Check sheet for the modelled part. Datum: model origin and axes. Units: mm. Face numbers are marked on the shaded views. A direction names the side the tool comes from. Round coordinates to 2 decimals unless told otherwise and drop trailing zeros. Loops run counter-clockwise (first coordinate to the right, second up) from the corner with the lowest first, then second, coordinate; pieces in that order, holes last. Notation, with made-up numbers: M -6,42 L 17,42 A25 ccw 17,63 Z; hole C 49,9.5 d6. An arc over 180 degrees is marked long. One line per question, with ' | ' between items. Start each with the question number.
(1) Section check C-C (y = 16.5). Record the boundary of the cut face in (x, z), and give its area (3 significant figures).
(2) Go/stop test with flat-tipped pins: P1, Ø0.9, axis at y = 39, z = 4, coming from the -X side; P2, Ø4, axis at y = 20, z = 3, coming from the +X side; P3, Ø1.5, axis at y = 24.5, z = 6.5, coming from the +X side. Record where each tip stops, or that it passes through.
(3) Section check B-B (x = 0). Record the boundary of the cut face in (y, z).
(4) Section check A-A (z = 0). Record the boundary of the cut face in (x, y), and give its area (3 significant figures).
(5) Section check D-D (y = 33). Record the boundary of the cut face in (x, z).
(6) Tool access check on the marked faces 4 and 5. Record the directions out of +Z, -Z, +X, -X, +Y, -Y that give a thin tool (end or side, any length) a straight path to the whole face; none if there is none.
(7) Thickness scan on probe 1 along Y at (x, z) = (6.5, -7.5); probe 2 along X at (y, z) = (12.5, -0.25); probe 3 along Y at (x, z) = (-0.75, -3.25). Record the ranges inside material, lowest first. Write a range as [from, to].
(8) Draft check along X on the marked faces 1, 2 and 3. Enter one of: +X half, -X half, draft (parallel to the pull), parting line (faces both ways), or undercut.
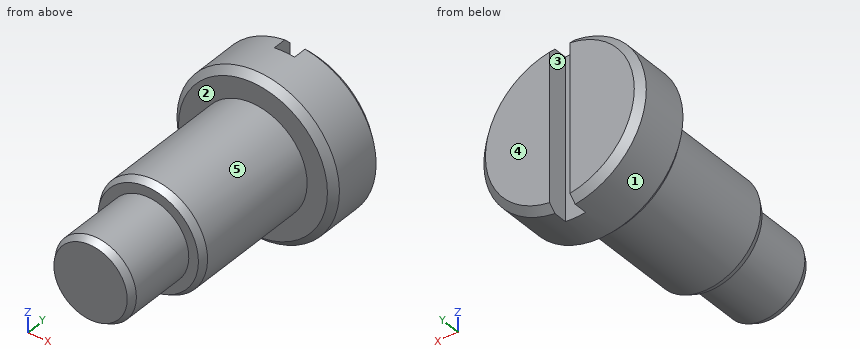
```python
from build123d import *
from OCP.BRepFilletAPI import BRepFilletAPI_MakeChamfer

# Parameters (mm, degrees)
CHAMFER1_SIZE      = 1
CHAMFER2_SIZE      = 1
CHAMFER2_SIZE2     = 0.577350269
SKETCH2_W          = 3
SKETCH2_H          = 30.588331256
CUT_EXTRUDE1_DEPTH = 3


with BuildPart() as part:
    # Sketch1 → Revolve1 (revolve)
    with BuildSketch(Plane.XY, mode=Mode.PRIVATE) as revolve1_sk:
        Polygon((0, 0), (0, 40), (12, 40), (12, 31), (8, 31), (8, 11), (6, 11), (6, 0), align=None)
    revolve(revolve1_sk.sketch.rotate(Axis((0, 0, 0), (0, 1, 0)), 90), axis=Axis((0, 0, 0), (0, 1, 0)))

    # Chamfer1
    chamfer1_edges = [part.edges().sort_by_distance(p)[0] for p in [
        (0, 31, 12),
        (0, 40, 12),
    ]]
    chamfer(chamfer1_edges, length=CHAMFER1_SIZE)

    # Chamfer2: one chamfer whose edges measure the first distance from different faces: ONE call of the kernel's chamfer builder (chamfer() names one face for all edges)
    chamfer2_edges_1 = [part.edges().sort_by_distance(p)[0] for p in [
        (0, 0, 6),
    ]]
    chamfer2_side_1 = [part.faces().sort_by_distance(p)[0] for p in [
        (0, 5.5, 6),
    ]]
    chamfer2_edges_2 = [part.edges().sort_by_distance(p)[0] for p in [
        (0, 11, 8),
    ]]
    chamfer2_side_2 = [part.faces().sort_by_distance(p)[0] for p in [
        (0, 21, 8),
    ]]
    chamfer2 = BRepFilletAPI_MakeChamfer(part.part.solid().wrapped)
    for e in chamfer2_edges_1:
        chamfer2.Add(CHAMFER2_SIZE, CHAMFER2_SIZE2, e.wrapped, chamfer2_side_1[0].wrapped)  # the first distance lies on this face
    for e in chamfer2_edges_2:
        chamfer2.Add(CHAMFER2_SIZE, CHAMFER2_SIZE2, e.wrapped, chamfer2_side_2[0].wrapped)  # the first distance lies on this face
    add(Compound.cast(chamfer2.Shape()), mode=Mode.REPLACE)

    # Sketch2 → Cut-Extrude1 (cut)
    with BuildSketch(Plane(origin=(0, 40, 0), x_dir=(1, 0, 0), z_dir=(0, 1, 0))):
        Rectangle(SKETCH2_W, SKETCH2_H)
    extrude(amount=-CUT_EXTRUDE1_DEPTH, mode=Mode.SUBTRACT)


solid = part.part
```
The answers:
1) outline: C 0,0 d16 | area: 201 mm²
2) P1: x = -11.46 | P2: x = 7.94 | P3: x = 5.56
3) outline: M 0,-5.42 L 1,-6 L 11,-6 L 11,-7.42 L 12,-8 L 31,-8 L 31,-11 L 32,-12 L 37,-12 L 37,12 L 32,12 L 31,11 L 31,8 L 12,8 L 11,7.42 L 11,6 L 1,6 L 0,5.42 Z
4) outline: M -12,32 L -11,31 L -8,31 L -8,12 L -7.42,11 L -6,11 L -6,1 L -5.42,0 L 5.42,0 L 6,1 L 6,11 L 7.42,11 L 8,12 L 8,31 L 11,31 L 12,32 L 12,39 L 11,40 L 1.5,40 L 1.5,37 L -1.5,37 L -1.5,40 L -11,40 L -12,39 Z | area: 656 mm²
5) outline: C 0,0 d24
6) face 4: +Z, -Z, +X, -X, +Y | face 5: -Y
7) probe 1: [31, 40] | probe 2: [-8, 8] | probe 3: [0, 37]
8) face 1: parting line | face 2: draft | face 3: undercut
